Can you work these out from the model? Positions are in its coordinate system, mm. Face numbers are marked on the shaded views. A direction names the side the tool comes from. Give positions to 0.01 mm unless a question says otherwise; leave off trailing zeros. Write each loop counter-clockwise with the first axis right and the second up, starting at its lowest first coordinate (ties: lowest second). Pieces come first, ordered by that corner, then holes.
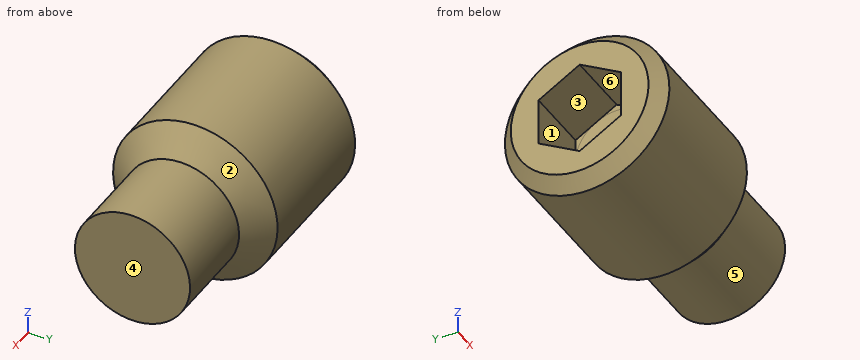
```python
from build123d import *

# Parameters (mm, degrees)
HEXAGONSOCKET_DEPTH = 4


with BuildPart() as part:
    # Sketch1 → Base (revolve)
    with BuildSketch(Plane.XY, mode=Mode.PRIVATE) as base_sk:
        Polygon((0, 0), (16, 0), (16, 3.5), (10.7, 3.5), (9.2, 5), (0.812, 5), (0, 4.188), align=None)
    revolve(base_sk.sketch.rotate(Axis((-1.968820569, 0, 0), (1, 0, 0)), 90), axis=Axis((-1.968820569, 0, 0), (1, 0, 0)))

    # Sketch2 → HexagonSocket (cut)
    with BuildSketch(Plane(origin=(0, -1.128463942, -0.35035393), x_dir=(0, 0, 1), z_dir=(-1, 0, 0))):
        Polygon((3.237105276, 1.128463942), (1.793729603, 3.628463942), (-1.093021743, 3.628463942), (-2.536397416, 1.128463942), (-1.093021743, -1.371536058), (1.793729603, -1.371536058), align=None)
    extrude(amount=-HEXAGONSOCKET_DEPTH, mode=Mode.SUBTRACT)

    # Sketch3 → Cut-Revolve1 (revolve, cut)
    with BuildSketch(Plane.XY, mode=Mode.PRIVATE) as cut_revolve1_sk:
        Polygon((4, 2.5), (4, 0), (4.8, 0), align=None)
    revolve(cut_revolve1_sk.sketch.rotate(Axis((-0.330994676, 0, 0), (1, 0, 0)), 90), axis=Axis((-0.330994676, 0, 0), (1, 0, 0)), mode=Mode.SUBTRACT)


solid = part.part
```
1) For pin 1 Ø3 at (x, z) = (11.5, -1.5) entering from -Y; pin 2 Ø1.5 at (x, z) = (6.5, -2) entering from +Y; pin 3 Ø1.5 at (y, z) = (-3.5, -3) entering from +X, each with a flat end and sliding along its axis, tell me the tip position at first contact or that it passes through.
Values follow:
pin 1: stops at y = -4
pin 2: stops at y = 4.84
pin 3: stops at x = 10.34
2) Suppose I cut it at B-B on x = 8.25. Write out the boundary of the cut face in (y, z), plus the area to 3 significant figures.
Values follow:
outline: circle Ø10 at (0, 0)
area: 78.5 mm2
3) Please list where these lines run through material, in increasing order: L1, parallel to Z at x = 3.25, y = -2; L2, parallel to Y at x = 4.5, z = -3.5; L3, parallel to Z at x = 13.25, y = 0.5.
Values follow:
L1: z = -4.58 to -1.73, 1.73 to 4.58
L2: y = -3.57 to 3.57
L3: z = -3.46 to 3.46
4) For the marked faces 1 and 2, which set-ups out of +Z, -Z, +X, -X, +Y, -Y let a thin tool reach every point of the face, with its end or its side?
Values follow:
face 1: -X
face 2: +X
5) Suppose I cut it at A-A on x = 4.5. Write out the boundary of the cut face in (y, z) (1 decimal), plus the area to 3 significant figures.
Values follow:
outline: circle Ø10 at (0, 0); hole circle Ø1.9 at (0, 0)
area: 75.8 mm2
6) If we mould it in two halves opening along Z, with no side actions, what happens to the marked faces 3, 4, 5 and 6? For each: +Z half, -Z half, draft (parallel to the pull), parting line (faces both ways), or undercut.
Values follow:
face 3: undercut
face 4: draft
face 5: parting line
face 6: undercut
